```python
from build123d import *

# Parameters (mm, degrees)
CHAMFER_1_SIZE           = 1.387
CUT_EXTRUDE_START        = -14.5
SKETCH_4_R               = 23.805
CUT_EXTRUDE_1_DEPTH      = 14.5
SKETCH_5_OUTSIDE_W       = 135.604
SKETCH_5_OUTSIDE_H       = 135.604
SKETCH_5_OUTSIDE_R       = 16.767
CUT_EXTRUDE_2_DEPTH      = 11.6
CUT_EXTRUDE_2_DRAFT      = -60
SKETCH_8_R               = 38.709
CUT_EXTRUDE_3_DEPTH      = 65.226413569
SKETCH_10_OUTSIDE_W      = 119.53
SKETCH_10_OUTSIDE_H      = 128.96
SKETCH_10_OUTSIDE_R      = 28.951662261
CUT_EXTRUDE_4_DEPTH      = 10
CUT_EXTRUDE_4_DRAFT      = -60
MIRROR_7_COPY_1_SKETCH_W = 135.604
MIRROR_7_COPY_1_SKETCH_H = 135.604
MIRROR_7_COPY_1_SKETCH_R = 16.767
MIRROR_7_COPY_1_DEPTH    = 11.6
MIRROR_7_COPY_1_DRAFT    = -60
MIRROR_7_COPY_2_SKETCH_W = 119.53
MIRROR_7_COPY_2_SKETCH_H = 128.96
MIRROR_7_COPY_2_SKETCH_R = 28.951662261
MIRROR_7_COPY_2_DEPTH    = 10
MIRROR_7_COPY_2_DRAFT    = -60


with BuildPart() as part:
    # 草图1 → 旋转1 (revolve)
    with BuildSketch(Plane.XY, mode=Mode.PRIVATE) as revolve_1_sk:
        Polygon((29, 20.7), (11.6, 20.7), (11.6, 23.805), (0, 23.805), (0, 27.324), (-11.6, 27.324), (-11.6, 20.7), (-29, 20.7), (-29, 14.477621389), (-11.6, 13.87), (11.6, 13.87), (29, 14.477621389), align=None)
    revolve(revolve_1_sk.sketch.rotate(Axis((0, 0, 0), (1, 0, 0)), 90), axis=Axis((0, 0, 0), (1, 0, 0)))

    # 倒角1
    chamfer_1_edges = [part.edges().sort_by_distance(p)[0] for p in [
        (-11.6, 0, -27.324),
        (11.6, 0, -23.805),
    ]]
    chamfer(chamfer_1_edges, length=CHAMFER_1_SIZE)

    # 草图3 → 旋转2 (revolve)
    with BuildSketch(Plane.XY, mode=Mode.PRIVATE) as revolve_2_sk:
        Polygon((-11.6, 27.324), (-11.6, 35.19), (11.6, 35.19), (11.6, 23.805), (0, 23.805), (0, 27.324), align=None)
    revolve(revolve_2_sk.sketch.rotate(Axis((0, 0, 0), (1, 0, 0)), 90), axis=Axis((0, 0, 0), (1, 0, 0)))

    # 草图4 → 切除-拉伸1 (cut)
    with BuildSketch(Plane(origin=(29, 0, 0), x_dir=(0, 0, -1), z_dir=(1, 0, 0)).offset(CUT_EXTRUDE_START)):
        with Locations(Location((0, 0, 0), (0, 0, 180))):
            Circle(SKETCH_4_R)
        Polygon((0, 20.7), (-17.926725858, 10.35), (-17.926725858, -10.35), (0, -20.7), (17.926725858, -10.35), (17.926725858, 10.35), align=None, mode=Mode.SUBTRACT)
    cut_extrude_1 = extrude(amount=CUT_EXTRUDE_1_DEPTH, mode=Mode.SUBTRACT)


with BuildPart() as cut_extrude_2_tool:
    # 草图5 outside → 切除-拉伸2 (with draft: the straight prism first)
    with BuildSketch(Plane(origin=(29, 0, 0), x_dir=(0, 0, -1), z_dir=(1, 0, 0))):
        Rectangle(SKETCH_5_OUTSIDE_W, SKETCH_5_OUTSIDE_H)
        Circle(SKETCH_5_OUTSIDE_R, mode=Mode.SUBTRACT)
    extrude(amount=-CUT_EXTRUDE_2_DEPTH)
    # 切除-拉伸2: the draft: its side faces are tilted about the plane it starts from
    cut_extrude_2_sides = [cut_extrude_2_tool.faces().sort_by_distance(p)[0] for p in [
        (23.2, -67.802, 0),
        (23.2, 0, -67.802),
        (23.2, 67.802, 0),
        (23.2, 0, 67.802),
        (23.2, 0, 16.767),
    ]]
    draft(cut_extrude_2_sides, Plane(origin=(29, 0, 0), x_dir=(0, 0, -1), z_dir=(1, 0, 0)), CUT_EXTRUDE_2_DRAFT)


with BuildPart() as part_1:
    add(part.part)

    # 切除-拉伸2: cut by cut_extrude_2_tool
    add(cut_extrude_2_tool.part, mode=Mode.SUBTRACT)

    # 草图6 → 旋转3 (revolve)
    with BuildSketch(Plane.XY, mode=Mode.PRIVATE) as revolve_3_sk:
        with BuildLine():
            Line((18.899592609, 14.124907391), (11.6, 14.124907391))
            Line((11.6, 14.124907391), (11.6, 21.4245))
            ThreePointArc((11.6, 21.4245), (13.738001175, 16.262908566), (18.899592609, 14.124907391))
        make_face()
    revolve_3 = revolve(revolve_3_sk.sketch.rotate(Axis((0, 0, 0), (1, 0, 0)), 120), axis=Axis((0, 0, 0), (1, 0, 0)))

    # 草图8 → 切除-拉伸3 (cut, through all)
    with BuildSketch(Plane(origin=(11.6, 0, 0), x_dir=(0, 0, -1), z_dir=(1, 0, 0))):
        Circle(SKETCH_8_R)
        Polygon((0, 35.19), (-30.475433959, 17.595), (-30.475433959, -17.595), (0, -35.19), (30.475433959, -17.595), (30.475433959, 17.595), align=None, mode=Mode.SUBTRACT)
    extrude(amount=-CUT_EXTRUDE_3_DEPTH, mode=Mode.SUBTRACT)


with BuildPart() as cut_extrude_4_tool:
    # 草图10 outside → 切除-拉伸4 (with draft: the straight prism first)
    with BuildSketch(Plane(origin=(11.6, 0, 0), x_dir=(0, 0, -1), z_dir=(1, 0, 0))):
        Rectangle(SKETCH_10_OUTSIDE_W, SKETCH_10_OUTSIDE_H)
        Circle(SKETCH_10_OUTSIDE_R, mode=Mode.SUBTRACT)
    extrude(amount=-CUT_EXTRUDE_4_DEPTH)
    # 切除-拉伸4: the draft: its side faces are tilted about the plane it starts from
    cut_extrude_4_sides = [cut_extrude_4_tool.faces().sort_by_distance(p)[0] for p in [
        (6.6, -64.48, 0),
        (6.6, 0, -59.765),
        (6.6, 64.48, 0),
        (6.6, 0, 59.765),
        (6.6, 0, 28.951662261),
    ]]
    draft(cut_extrude_4_sides, Plane(origin=(11.6, 0, 0), x_dir=(0, 0, -1), z_dir=(1, 0, 0)), CUT_EXTRUDE_4_DRAFT)


with BuildPart() as part_2:
    add(part_1.part)

    # 切除-拉伸4: cut by cut_extrude_4_tool
    add(cut_extrude_4_tool.part, mode=Mode.SUBTRACT)

    # 镜向7: 切除-拉伸1, 旋转3 across plane
    add(cut_extrude_1.mirror(Plane(origin=(0, 0, 0), x_dir=(0, 0, 1), z_dir=(1, 0, 0))), mode=Mode.SUBTRACT)
    add(revolve_3.mirror(Plane(origin=(0, 0, 0), x_dir=(0, 0, 1), z_dir=(1, 0, 0))))


with BuildPart() as mirror_7_copy_1_tool:
    # 镜向7 copy 1 sketch → 镜向7 copy 1 (with draft: the straight prism first)
    with BuildSketch(Plane(origin=(-29, 0, 0), x_dir=(0, 0, -1), z_dir=(-1, 0, 0))):
        Rectangle(MIRROR_7_COPY_1_SKETCH_W, MIRROR_7_COPY_1_SKETCH_H)
        Circle(MIRROR_7_COPY_1_SKETCH_R, mode=Mode.SUBTRACT)
    extrude(amount=-MIRROR_7_COPY_1_DEPTH)
    # 镜向7 copy 1: the draft: its side faces are tilted about the plane it starts from
    mirror_7_copy_1_sides = [mirror_7_copy_1_tool.faces().sort_by_distance(p)[0] for p in [
        (-23.2, -67.802, 0),
        (-23.2, 0, -67.802),
        (-23.2, 67.802, 0),
        (-23.2, 0, 67.802),
        (-23.2, 0, 16.767),
    ]]
    draft(mirror_7_copy_1_sides, Plane(origin=(-29, 0, 0), x_dir=(0, 0, -1), z_dir=(-1, 0, 0)), MIRROR_7_COPY_1_DRAFT)


with BuildPart() as part_3:
    add(part_2.part)

    # 镜向7 copy 1: cut by mirror_7_copy_1_tool
    add(mirror_7_copy_1_tool.part, mode=Mode.SUBTRACT)


with BuildPart() as mirror_7_copy_2_tool:
    # 镜向7 copy 2 sketch → 镜向7 copy 2 (with draft: the straight prism first)
    with BuildSketch(Plane(origin=(-11.6, 0, 0), x_dir=(0, 0, -1), z_dir=(-1, 0, 0))):
        Rectangle(MIRROR_7_COPY_2_SKETCH_W, MIRROR_7_COPY_2_SKETCH_H)
        Circle(MIRROR_7_COPY_2_SKETCH_R, mode=Mode.SUBTRACT)
    extrude(amount=-MIRROR_7_COPY_2_DEPTH)
    # 镜向7 copy 2: the draft: its side faces are tilted about the plane it starts from
    mirror_7_copy_2_sides = [mirror_7_copy_2_tool.faces().sort_by_distance(p)[0] for p in [
        (-6.6, -64.48, 0),
        (-6.6, 0, -59.765),
        (-6.6, 64.48, 0),
        (-6.6, 0, 59.765),
        (-6.6, 0, 28.951662261),
    ]]
    draft(mirror_7_copy_2_sides, Plane(origin=(-11.6, 0, 0), x_dir=(0, 0, -1), z_dir=(-1, 0, 0)), MIRROR_7_COPY_2_DRAFT)


with BuildPart() as part_4:
    add(part_3.part)

    # 镜向7 copy 2: cut by mirror_7_copy_2_tool
    add(mirror_7_copy_2_tool.part, mode=Mode.SUBTRACT)


solid = part_4.part
```
Design review of the part built by this model. Coordinates are the model's own, in mm. A direction names the side the tool comes from. Give positions to 0.01 mm unless a question says otherwise; leave off trailing zeros. Write each loop counter-clockwise with the first axis right and the second up, starting at its lowest first coordinate (ties: lowest second). Pieces come first, ordered by that corner, then holes. Notation, with made-up numbers: (10.5, 63) -> (20.5, 63) arc R18 ccw to (20.5, 72) -> close; hole circle Ø5 at (-11, 6). An arc over 180 degrees is marked (long way). Answer in a Markdown table with one row per item.
(1) Clearance check with flat-ended pins moving along their axes: pin 1 (7 mm diameter, centred on x = -21, y = 2.5, fed in from +Z); pin 2 (3 mm diameter, centred on y = 14.5, z = 23, fed in from -X); pin 3 (1.4 mm diameter, centred on y = -0.5, z = -20, fed in from +X). State where each tip first meets the part, or that it passes through.
Results:
| item | result |
|---|---|
| pin 1 | z = 17.93 |
| pin 2 | x = -11.6 |
| pin 3 | x = 14.5 |
(2) For faces 4 (the flat face through (14.5, -16, 10)), 5 (the flat face through (11.6, 18, -12)), 6 (the flat face through (-21, 0, 17.927)), list the 3-axis set-ups (+Z, -Z, +X, -X, +Y, -Y) from which the entire face can be reached by the end or side of a thin tool; tool diameter is ignored.
Results:
| item | result |
|---|---|
| face 4 | +Z, +X, -Y |
| face 5 | +X |
| face 6 | +Z, -X, +Y, -Y |
(3) Consider section A-A (x = -18). State the section outline as (y, z) points.
Results:
| item | result |
|---|---|
| outline | (-20.7, 0) -> (-10.35, -17.93) -> (10.35, -17.93) -> (20.7, 0) -> (10.35, 17.93) -> (-10.35, 17.93) -> close; hole circle Ø28.19 at (0, 0) |
(4) To check wall thickness, follow probe 1 along Y at (x, z) = (5, 0); probe 2 along Y at (x, z) = (-11.3, 0); probe 3 along Y at (x, z) = (11.25, 0) (3 decimals). State the ranges of each line that lie inside material, in increasing order.
Results:
| item | result |
|---|---|
| probe 1 | -35.19 to -13.87, 13.87 to 35.19 |
| probe 2 | -29.47 to -27.32, -26.24 to -13.87, 13.87 to 26.24, 27.32 to 29.47 |
| probe 3 | -29.558 to -23.805, -22.768 to -13.87, 13.87 to 22.768, 23.805 to 29.558 |
(5) Mouldability with a two-part tool opening along Y and no side actions: class faces 1 (the flat face through (14.5, 0, 19)), 2 (the flat face through (21.32, -15.45, 9.09)), 3 (the cylindrical face through (10.897, -7.15, 22.706)) as +Y half, -Y half, draft (parallel to the pull), parting line (faces both ways), or undercut.
Results:
| item | result |
|---|---|
| face 1 | draft |
| face 2 | -Y half |
| face 3 | undercut |
(6) Consider section B-B (x = 16). State the section outline as (y, z) points, then the cut area to 3 significant figures.
Results:
| item | result |
|---|---|
| outline | (-20.7, 0) -> (-10.35, -17.93) -> (10.35, -17.93) -> (20.7, 0) -> (10.35, 17.93) -> (-10.35, 17.93) -> close; hole circle Ø28.05 at (0, 0) |
| area | 495 mm2 |
